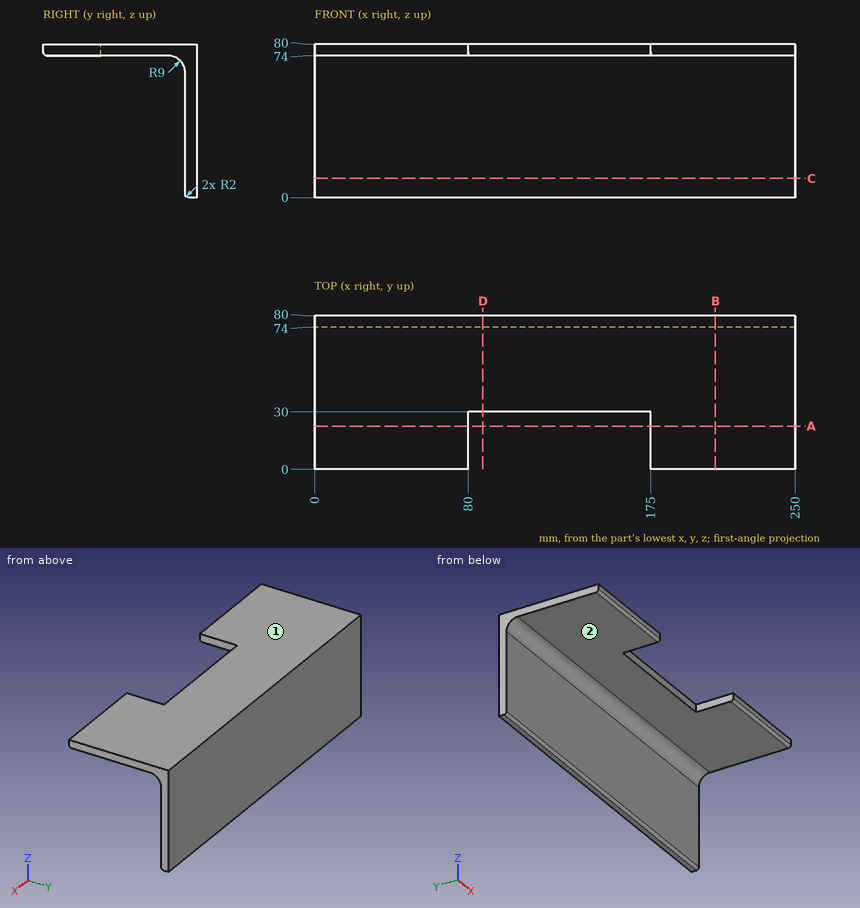
Geometry: see drawing. Coordinates: mm, zero at the bounding-box minimum. A direction names the side the tool comes from. Coordinates: 2 decimals unless noted, no trailing zeros. Order: outer loops, then holes, each group sorted by start corner. A loop starts at its lowest first (then second) coordinate and runs counter-clockwise, first axis right, second up. Notation, with made-up numbers: (44, 5.25) - (53, 5.25) arc R20 ccw to (53, 22.25) - close; hole circle Ø10 at (27, 83.5). An arc over 180 degrees is marked (long way). Return JSON: item names as keys, results as strings.
Q1. Cut plane A-A (y = 22.5). Return loops of the section in (x, z).
The answers:
{"outline": "(0, 74) - (80, 74) - (80, 80) - (0, 80) - close; (175, 74) - (250, 74) - (250, 80) - (175, 80) - close"}
Q2. Cut plane C-C (z = 10). Return loops of the section in (x, y).
The answers:
{"outline": "(0, 74) - (250, 74) - (250, 80) - (0, 80) - close"}
Q3. Access query for the marked faces 1 and 2. Directions: +Z, -Z, +X, -X, +Y, -Y. A direction counts if a zero-diameter tool reaches every point of the face in a straight line with its end or side. Return the directions, or none.
The answers:
{"face 1": "+Z, +X, -X, +Y, -Y", "face 2": "-Z, +X, -X, -Y"}
Q4. Cut plane B-B (x = 208.5). Return loops of the section in (y, z), then the cut area to 3 significant figures.
The answers:
{"outline": "(0, 76) arc R2 ccw to (2, 74) - (65, 74) arc R9 cw to (74, 65) - (74, 2) arc R2 ccw to (76, 0) - (80, 0) - (80, 80) - (0, 80) - close", "area": "940 mm2"}
Q5. Ray query, probe 1 along X at (y, z) = (25.5, 75.5); probe 2 along Y at (x, z) = (224.5, 50.5). Return the intervals inside material, ascending.
The answers:
{"probe 1": "x = 0 to 80, 175 to 250", "probe 2": "y = 74 to 80"}
Q6. Cut plane D-D (x = 87.5). Return loops of the section in (y, z).
The answers:
{"outline": "(30, 74) - (65, 74) arc R9 cw to (74, 65) - (74, 2) arc R2 ccw to (76, 0) - (80, 0) - (80, 80) - (30, 80) - close"}
Q7. First-contact query: pin 1 (10 mm diameter, centred on x = 115, y = 29.5, fed in from -Z); pin 2 (5 mm diameter, centred on x = 150.5, z = 77.5, fed in from -Y); pin 3 (19 mm diameter, centred on x = 161, z = 19.5, fed in from -Y); pin 4 (6.5 mm diameter, centred on y = 17, z = 77.5, fed in from -X). Flat tips, straight axial feed; report the tip coordinate or a pass-through.
The answers:
{"pin 1": "stops at z = 74", "pin 2": "stops at y = 30", "pin 3": "stops at y = 74", "pin 4": "stops at x = 0"}
